For this review, take the finished solid that the model builds, in its own axes (mm). Coordinates: 2 decimals unless noted, no trailing zeros. Order: outer loops, then holes, each group sorted by start corner. A loop starts at its lowest first (then second) coordinate and runs counter-clockwise, first axis right, second up. Notation, with made-up numbers: (63, -39) -> (109, -39) arc R10 cw to (109, -25) -> close; hole circle Ø10 at (-12, 47.5). An arc over 180 degrees is marked (long way). Write item = value, one per line. Start each with the question number.
1) Consider section B-B on z = 5.25. Give the boundary of the cut face in (x, y).
2) Wall thickness on probe 1 along Y at (x, z) = (0, 3.5); probe 2 along Y at (x, z) = (-2, 4.25): over which ranges is each line inside the solid? List them lowest first. Write a range as [from, to].
3) Draft analysis for pull direction Y (two halves, no side actions). For faces 1 (the face through (0.358, -28.773, 3.451)), 2 (the face through (0, -37.5, 3)), 3 (the face through (0, 1, 0)), state which applies: +Y half, -Y half, draft (parallel to the pull), parting line (faces both ways), or undercut.
4) Consider section C-C on y = 31.5. Give the boundary of the cut face in (x, z).
5) Insertion check: pin 1 Ø3 at (x, y) = (-3.5, -20.5) entering from -Z. The pin has a flat end and moves straight along its axis. Give the tip position at first contact, or say it passes through.
6) Consider section A-A on x = 0. Give the boundary of the cut face in (y, z).
from build123d import *

# Parameters (mm, degrees)
SKETCH1_W            = 16
SKETCH1_H            = 75
BOSS_EXTRUDE1_DEPTH  = 7
CHAMFER5_SIZE        = 1
M5_CLEARANCE_HOLE1_D = 5.5


with BuildPart() as part:
    # Sketch1 → Boss-Extrude1 (new body)
    with BuildSketch(Plane.XY):
        Rectangle(SKETCH1_W, SKETCH1_H)
    extrude(amount=BOSS_EXTRUDE1_DEPTH)

    # Chamfer5
    chamfer5_edges = [part.edges().sort_by_distance(p)[0] for p in [
        (8, -37.5, 3.5),
        (-8, -37.5, 3.5),
        (-8, 37.5, 3.5),
        (8, 37.5, 3.5),
    ]]
    chamfer(chamfer5_edges, length=CHAMFER5_SIZE)

    # M5 Clearance Hole1 (through all)
    with Locations(Plane.XY.offset(7)):
        with Locations((0, 31.5), (0, -31.5)):
            Hole(M5_CLEARANCE_HOLE1_D / 2)


solid = part.part
Answer sheet:
q1.outline = (-8, -36.5) -> (-7, -37.5) -> (7, -37.5) -> (8, -36.5) -> (8, 36.5) -> (7, 37.5) -> (-7, 37.5) -> (-8, 36.5) -> close; hole circle Ø5.5 at (0, -31.5); hole circle Ø5.5 at (0, 31.5)
q2.probe_1 = [-37.5, -34.25], [-28.75, 28.75], [34.25, 37.5]
q2.probe_2 = [-37.5, -33.39], [-29.61, 29.61], [33.39, 37.5]
q3.face_1 = undercut
q3.face_2 = -Y half
q3.face_3 = draft
q4.outline = (-8, 0) -> (-2.75, 0) -> (-2.75, 7) -> (-8, 7) -> close; (2.75, 0) -> (8, 0) -> (8, 7) -> (2.75, 7) -> close
q5.pin_1 = 0
q6.outline = (-37.5, 0) -> (-34.25, 0) -> (-34.25, 7) -> (-37.5, 7) -> close; (-28.75, 0) -> (28.75, 0) -> (28.75, 7) -> (-28.75, 7) -> close; (34.25, 0) -> (37.5, 0) -> (37.5, 7) -> (34.25, 7) -> close
